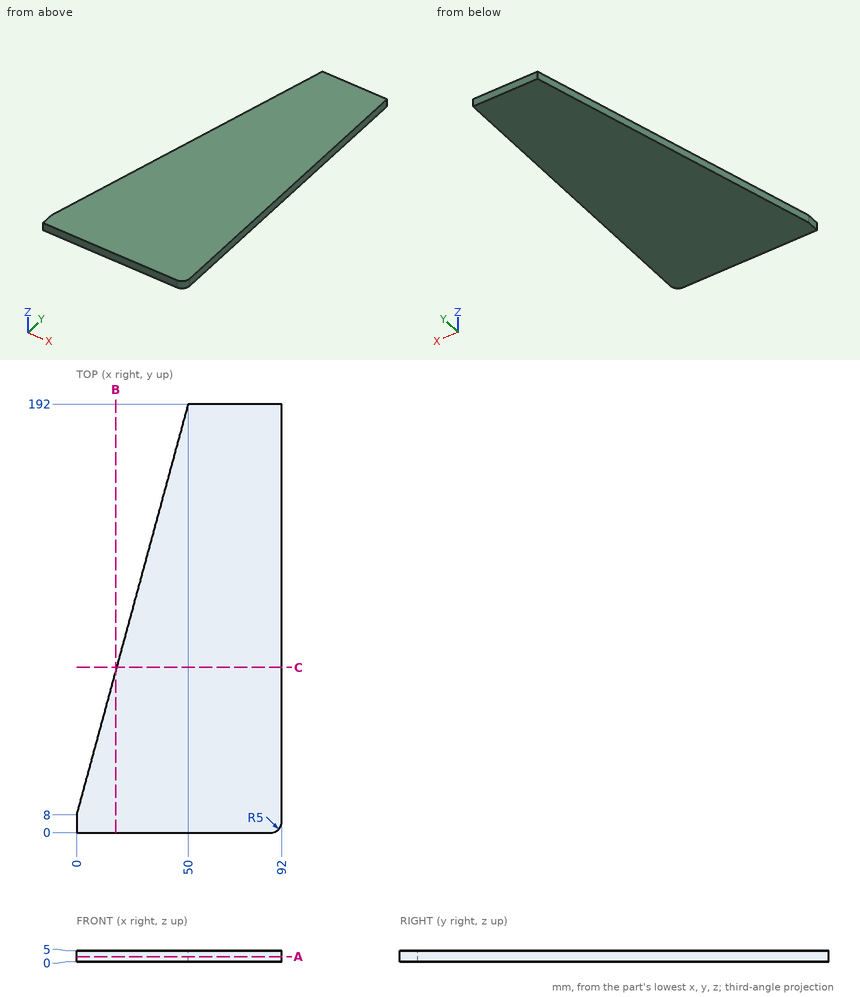
Geometry: see drawing. Coordinates: mm, zero at the bounding-box minimum. Give positions to 0.01 mm unless a question says otherwise; leave off trailing zeros. Order: outer loops, then holes, each group sorted by start corner. A loop starts at its lowest first (then second) coordinate and runs counter-clockwise, first axis right, second up. Notation, with made-up numbers: (-17, 89) - (28, 89) arc R25 ccw to (28, 125) - close; hole circle Ø3 at (16.5, 62). An arc over 180 degrees is marked (long way). One line per item, written item: value.
1. Cut plane A-A, the plane z = 2.3. Output: boundary loops of the cut face in (x, y).
Determined:
outline: (0, 0) - (87, 0) arc R5 ccw to (92, 5) - (92, 192) - (50, 192) - (0, 8) - close
2. Line query: probe 1 along X at (y, z) = (177, 3.75); probe 2 along X at (y, z) = (46, 3.75); probe 3 along Y at (x, z) = (88, 0.2). Output: solid intervals per line, ascending.
Determined:
probe 1: 45.92 to 92
probe 2: 10.33 to 92
probe 3: 0.1 to 192
3. Cut plane B-B, the plane x = 17.5. Output: boundary loops of the cut face in (y, z), and give its area (3 significant figures).
Determined:
outline: (0, 0) - (72.4, 0) - (72.4, 5) - (0, 5) - close
area: 362 mm2
4. Pin query (flat end, axial travel): pin 1 Ø3 at (x, y) = (79.5, 23) entering from -Z; pin 2 Ø8 at (x, y) = (25, 120.5) entering from -Z; pin 3 Ø3 at (y, z) = (40, 1) entering from -X. Return the tip coordinate at first contact, or that it passes through.
Determined:
pin 1: z = 0
pin 2: through
pin 3: x = 8.29
5. Cut plane C-C, the plane y = 74. Output: boundary loops of the cut face in (x, z).
Determined:
outline: (17.93, 0) - (92, 0) - (92, 5) - (17.93, 5) - close
